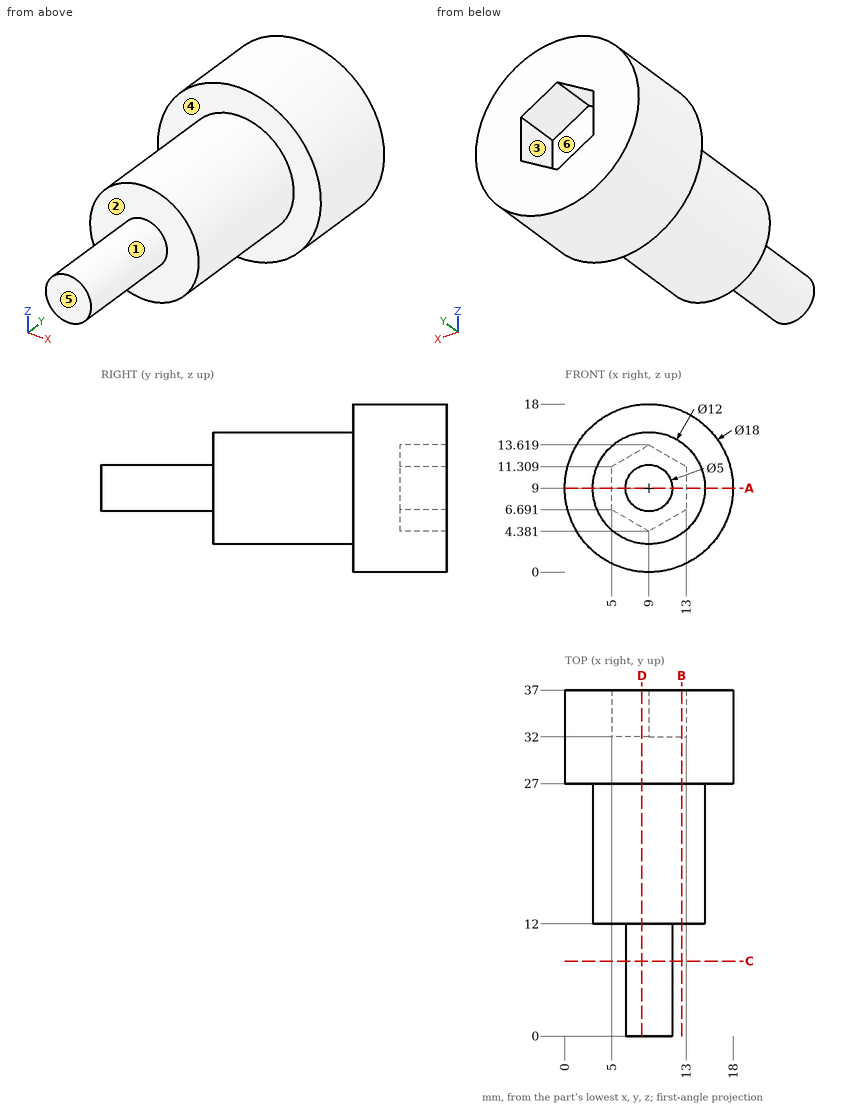
Geometry check sheet. Reference: drawing and pictorial views, mm from the part's lowest x, y, z. A direction names the side the tool comes from. Give positions to 0.01 mm unless a question says otherwise; leave off trailing zeros. Loops run counter-clockwise (first coordinate to the right, second up) from the corner with the lowest first, then second, coordinate; pieces in that order, holes last.
1. Section check D-D, the plane x = 8.25. Enter the section's corners in (y, z) (1 decimal).
2. Mould release check, pull along Z, two halves, no side actions. Record for the marked faces 1, 2 and 3: released by +Z, released by -Z, zero draft, split by the parting line, or undercut.
3. Thickness scan on line 1 (Y direction, x = 10, z = 10); line 2 (Y direction, x = 11.75, z = 1.25); line 3 (X direction, y = 32.5, z = 5.25) (1 decimal). Record the ranges inside material, lowest first.
4. Section check A-A, the plane z = 9. Enter the section's corners in (x, y).
5. Section check B-B, the plane x = 12.5. Enter the section's corners in (y, z).
6. Set-up check for the marked faces 4, 5 and 6: record each of +Z, -Z, +X, -X, +Y, -Y from which the full face is reachable in a straight line by a thin tool's end or side.
7. Go/stop test with flat-tipped pins: pin 1 Ø1 at (x, y) = (3, 21) entering from -Z (1 decimal); pin 2 Ø9 at (x, z) = (11, 8.5) entering from +Y; pin 3 Ø3 at (x, y) = (6.5, 19) entering from -Z; pin 4 Ø8 at (x, y) = (6, 19.5) entering from +Z. Record where each tip stops, or that it passes through.
8. Section check C-C, the plane y = 8. Enter the section's corners in (x, z).
Geometry says:
1. outline: (0, 6.6) - (12, 6.6) - (12, 3) - (27, 3) - (27, 0) - (37, 0) - (37, 4.8) - (32, 4.8) - (32, 13.2) - (37, 13.2) - (37, 18) - (27, 18) - (27, 15) - (12, 15) - (12, 11.4) - (0, 11.4) - close
2. face 1: split by the parting line
2. face 2: zero draft
2. face 3: undercut
3. line 1: y = 0 to 32
3. line 2: y = 27 to 37
3. line 3: x = 0.8 to 7.5, 10.5 to 17.2
4. outline: (0, 27) - (3, 27) - (3, 12) - (6.5, 12) - (6.5, 0) - (11.5, 0) - (11.5, 12) - (15, 12) - (15, 27) - (18, 27) - (18, 37) - (13, 37) - (13, 32) - (5, 32) - (5, 37) - (0, 37) - close
5. outline: (12, 4.13) - (27, 4.13) - (27, 0.71) - (37, 0.71) - (37, 6.4) - (32, 6.4) - (32, 11.6) - (37, 11.6) - (37, 17.29) - (27, 17.29) - (27, 13.87) - (12, 13.87) - close
6. face 4: -Y
6. face 5: +Z, -Z, +X, -X, -Y
6. face 6: +Y
7. pin 1: stops at z = 6.6
7. pin 2: stops at y = 37
7. pin 3: stops at z = 3.08
7. pin 4: stops at z = 15
8. outline: circle Ø5 at (9, 9)
